Geometry check sheet. Reference: the model listing, model coordinates, mm. A direction names the side the tool comes from. Coordinates: 2 decimals unless noted, no trailing zeros. Loops run counter-clockwise (first coordinate to the right, second up) from the corner with the lowest first, then second, coordinate; pieces in that order, holes last. Notation, with made-up numbers: (-31, 37) - (7, 37) arc R18 cw to (7, 66) - close; hole circle Ø1 at (6, -11.75). An arc over 180 degrees is marked (long way). Write each question's results on one line, items separated by ' | '. Start each with the question number.
(1) Access from +Z, -Z, +X, -X, +Y, -Y to the whole of each face (thin tool, end or side, straight path). Record for faces 1 (the face through (0, 0, 8.5)), 2 (the face through (1, -1, 3.5)).
(2) Sectioned sample at A-A (y = 0). Enter the section's corners in (x, z), plus the area to 3 significant figures.
(3) Sectioned sample at C-C (z = 3.25). Enter the section's corners in (x, y).
(4) Material ranges on probe 1 along Y at (x, z) = (-0.6, -3); probe 2 along Z at (x, y) = (-0.2, -1.3); probe 3 along Y at (x, z) = (0.8, -1.75), recorded low to high.
(5) Go/stop test with flat-tipped pins: pin 1 Ø1 at (x, y) = (-1, -1.5) entering from -Z; pin 2 Ø2 at (y, z) = (-1, 0) entering from +X. Record where each tip stops, or that it passes through.
from build123d import *

# Parameters (mm, degrees)
SKETCH1_R           = 1
BOSS_EXTRUDE1_DEPTH = 8.5
SKETCH2_R           = 2
BOSS_EXTRUDE2_DEPTH = 5
CHAMFER1_SIZE       = 0.2


with BuildPart() as part:
    # Sketch1 → Boss-Extrude1 (new, symmetric)
    with BuildSketch(Plane.XY):
        Circle(SKETCH1_R)
    extrude(amount=BOSS_EXTRUDE1_DEPTH, both=True)

    # Sketch2 → Boss-Extrude2 (add)
    with BuildSketch(Plane.XY.offset(8.5)):
        Circle(SKETCH2_R)
    extrude(amount=-BOSS_EXTRUDE2_DEPTH)

    # Chamfer1
    chamfer1_edges = [part.edges().sort_by_distance(p)[0] for p in [
        (-1, 0, -8.5),
        (-2, 0, 8.5),
        (-2, 0, 3.5),
    ]]
    chamfer(chamfer1_edges, length=CHAMFER1_SIZE)


solid = part.part
Outcome:
1) face 1: +Z, +X, -X, +Y, -Y | face 2: -Z
2) outline: (-2, 3.7) - (-1.8, 3.5) - (-1, 3.5) - (-1, -8.3) - (-0.8, -8.5) - (0.8, -8.5) - (1, -8.3) - (1, 3.5) - (1.8, 3.5) - (2, 3.7) - (2, 8.3) - (1.8, 8.5) - (-1.8, 8.5) - (-2, 8.3) - close | area: 43.9 mm2
3) outline: circle Ø2 at (0, 0)
4) probe 1: y = -0.8 to 0.8 | probe 2: z = 3.5 to 8.5 | probe 3: y = -0.6 to 0.6
5) pin 1: stops at z = 3.5 | pin 2: stops at x = 1
